from build123d import *

# Parameters (mm, degrees)
EXTRUDE_1_DEPTH              = 5
HOLE_WIZARD_8_5_8_5_1_D      = 8.5
PATTERN_LINEAR_1_COUNT       = 2
PATTERN_LINEAR_1_PITCH       = 40
MIRROR_1_COPY_1_D            = 8.5
CUT_EXTRUDE_1_DEPTH          = 10
HOLE_WIZARD_5_5_5_5_1_REACH  = 186.035
HOLE_WIZARD_5_5_5_5_1_BORE_R = 2.75
CHAMFER_1_SIZE               = 5


with BuildPart() as part:
    # 草图2 → 凸台-拉伸1 (new, symmetric)
    with BuildSketch(Plane.XY):
        with BuildLine():
            Line((-60, 38), (90, 38))
            Line((90, 38), (90, -38))
            Line((90, -38), (-90, -38))
            Line((-90, -38), (-90, 8))
            ThreePointArc((-90, 8), (-81.213203436, 29.213203436), (-60, 38))
        make_face()
    extrude(amount=EXTRUDE_1_DEPTH, both=True)

    # Ø8.5 (8.5) 直径孔1 (through all)
    with Locations(Plane.XY.offset(5)):
        with Locations((75, 20)):
            hole_wizard_8_5_8_5_1 = Hole(HOLE_WIZARD_8_5_8_5_1_D / 2)

    # 阵列(线性)1: Ø8.5 (8.5) 直径孔1 ×2
    with Locations(*[(-i * PATTERN_LINEAR_1_PITCH, 0, 0) for i in range(1, PATTERN_LINEAR_1_COUNT)]):
        add(hole_wizard_8_5_8_5_1, mode=Mode.SUBTRACT)

    # 镜向1: Ø8.5 (8.5) 直径孔1 across plane
    add(hole_wizard_8_5_8_5_1.mirror(Plane.ZX), mode=Mode.SUBTRACT)

    # 镜向1 copy 1 (through all)
    with Locations(Plane(origin=(-40, 0, 5), x_dir=(1, 0, 0), z_dir=(0, 0, 1))):
        with Locations((75, -20)):
            Hole(MIRROR_1_COPY_1_D / 2)

    # 草图5 → 切除-拉伸1 (cut)
    with BuildSketch(Plane.XY.offset(5)):
        with BuildLine():
            Line((-69, 6.5), (-34, 6.5))
            ThreePointArc((-34, 6.5), (-27, -0.5), (-34, -7.5))
            Line((-34, -7.5), (-69, -7.5))
            ThreePointArc((-69, -7.5), (-76, -0.5), (-69, 6.5))
        make_face()
    extrude(amount=-CUT_EXTRUDE_1_DEPTH, mode=Mode.SUBTRACT)

    # Ø5.5 (5.5) 直径孔1 bore → Ø5.5 (5.5) 直径孔1 (cut, up to next)
    with BuildSketch(Plane.ZY.offset(90), mode=Mode.PRIVATE) as hole_wizard_5_5_5_5_1_sk1:
        with Locations((0, -0.5)):
            Circle(HOLE_WIZARD_5_5_5_5_1_BORE_R)
    hole_wizard_5_5_5_5_1_tool1 = extrude(hole_wizard_5_5_5_5_1_sk1.sketch, amount=-HOLE_WIZARD_5_5_5_5_1_REACH, mode=Mode.PRIVATE) & part.part
    add(hole_wizard_5_5_5_5_1_tool1.solids().sort_by_distance((-90, -0.5, 0))[0], mode=Mode.SUBTRACT)

    # 倒角1
    chamfer_1_edges = [part.edges().sort_by_distance(p)[0] for p in [
        (90, -38, 0),
        (-90, -38, 0),
        (90, 38, 0),
    ]]
    chamfer(chamfer_1_edges, length=CHAMFER_1_SIZE)


solid = part.part
Check sheet for the modelled part. Datum: model origin and axes. Units: mm. A direction names the side the tool comes from. Round coordinates to 2 decimals unless told otherwise and drop trailing zeros. Loops run counter-clockwise (first coordinate to the right, second up) from the corner with the lowest first, then second, coordinate; pieces in that order, holes last. Notation, with made-up numbers: M 83,-32 L 98,-32 A14 cw 98,-14 Z; hole C 11,20 d2. An arc over 180 degrees is marked long. One line per item, written item: value.
(1) Release check for a two-part mould opening along X. For faces 1 (the face through (87, -36, 0)), 2 (the face through (-82.82, 1.359, -2.027)), 3 (the face through (-75.524, -3.038, 2.292)) record: +X half, -X half, draft (parallel to the pull), parting line (faces both ways), or undercut.
Computed values:
face 1: +X half
face 2: draft
face 3: undercut
(2) Sectioned sample at A-A, the plane z = 0. Record the cut outline in (x, y), then the cut area to 3 significant figures.
Computed values:
outline: M -90,-33 L -85,-38 L 85,-38 L 90,-33 L 90,33 L 85,38 L -60,38 A30 ccw -90,8 L -90,2.25 L -75.44,2.25 A7 cw -69,6.5 L -34,6.5 A7 cw -34,-7.5 L -69,-7.5 A7 cw -75.44,-3.25 L -90,-3.25 Z; hole C 35,-20 d8.5; hole C 35,20 d8.5; hole C 75,-20 d8.5; hole C 75,20 d8.5
area: 12,500 mm^2
(3) Access from +Z, -Z, +X, -X, +Y, -Y to the whole of each face (thin tool, end or side, straight path). Record for faces 4 (the face through (1, -38, 0)), 5 (the face through (-27, -0.35, 0.07)).
Computed values:
face 4: +Z, -Z, +X, -X, -Y
face 5: +Z, -Z
(4) Thickness scan on line 1 (Y direction, x = 34.5, z = -2.5); line 2 (Y direction, x = 72, z = -3); line 3 (Z direction, x = -81.25, y = -0.5). Record the ranges inside material, lowest first.
Computed values:
line 1: y = -38 to -24.22, -15.78 to 15.78, 24.22 to 38
line 2: y = -38 to -23.01, -16.99 to 16.99, 23.01 to 38
line 3: z = -5 to -2.75, 2.75 to 5
(5) Depth check by flat-ended pin: pin 1 Ø7.5 at (x, y) = (35, -20) entering from -Z. Enter the tip coordinate at first touch or a pass-through.
Computed values:
pin 1: passes through
(6) Sectioned sample at D-D, the plane y = -20. Record the cut outline in (x, z), then the cut area to 3 significant figures.
Computed values:
outline: M -90,-5 L 30.75,-5 L 30.75,5 L -90,5 Z; M 39.25,-5 L 70.75,-5 L 70.75,5 L 39.25,5 Z; M 79.25,-5 L 90,-5 L 90,5 L 79.25,5 Z
area: 1,630 mm^2
(7) Sectioned sample at B-B, the plane x = -37. Record the cut outline in (y, z).
Computed values:
outline: M -38,-5 L -7.5,-5 L -7.5,5 L -38,5 Z; M 6.5,-5 L 38,-5 L 38,5 L 6.5,5 Z
(8) Sectioned sample at C-C, the plane y = -0.5. Record the cut outline in (x, z), then the cut area to 3 significant figures.
Computed values:
outline: M -90,-5 L -76,-5 L -76,-2.75 L -90,-2.75 Z; M -90,2.75 L -76,2.75 L -76,5 L -90,5 Z; M -27,-5 L 90,-5 L 90,5 L -27,5 Z
area: 1,230 mm^2
